from build123d import *

# Parameters (mm, degrees)
SKETCH1_R           = 6
BOSS_EXTRUDE1_DEPTH = 5
SKETCH2_R           = 4
BOSS_EXTRUDE2_DEPTH = 1
SKETCH3_R           = 3
CUT_EXTRUDE1_DEPTH  = 11.392304845
CHAMFER1_SIZE       = 0.2


with BuildPart() as part:
    # Sketch1 → Boss-Extrude1 (new body)
    with BuildSketch(Plane.XY):
        Circle(SKETCH1_R)
    extrude(amount=BOSS_EXTRUDE1_DEPTH)

    # Sketch2 → Boss-Extrude2 (add)
    with BuildSketch(Plane.XY.offset(5)):
        Circle(SKETCH2_R)
    extrude(amount=BOSS_EXTRUDE2_DEPTH)

    # Sketch3 → Cut-Extrude1 (cut, through all)
    with BuildSketch(Plane.XY.offset(6)):
        Circle(SKETCH3_R)
    extrude(amount=-CUT_EXTRUDE1_DEPTH, mode=Mode.SUBTRACT)

    # Chamfer1
    chamfer1_edges = [part.edges().sort_by_distance(p)[0] for p in [
        (-6, 0, 0),
        (-6, 0, 5),
    ]]
    chamfer(chamfer1_edges, length=CHAMFER1_SIZE)

    # Sketch4 → M3 Tapped Hole1 (revolve, cut)
    with BuildSketch(Plane(origin=(0, 0, 2.5), x_dir=(0, 0, -1), z_dir=(1, 0, 0))):
        Polygon((0, 0), (0, 8.251075774), (1.25, 7.5), (1.25, 0), align=None)
    revolve(axis=Axis((0, -6.35, 2.5), (0, 1, 0)), mode=Mode.SUBTRACT)


solid = part.part
Source: CAD feature listing. Evaluate the final solid. Frame: model axes, mm. A direction names the side the tool comes from. Give positions to 0.01 mm unless a question says otherwise; leave off trailing zeros. Loops run counter-clockwise (first coordinate to the right, second up) from the corner with the lowest first, then second, coordinate; pieces in that order, holes last. Notation, with made-up numbers: (36, 64) -> (87, 64) arc R10 ccw to (87, 72) -> close; hole circle Ø4 at (2.25, 86.25). An arc over 180 degrees is marked (long way). Use a Markdown table: item, result. Add a question column.
1) Reachability of faces 4 (the face through (-1.24, 4.34, 2.66)), 5 (the face through (-0.867, -3.905, 5.493)), 6 (the face through (1, 3, 6)) from +Z, -Z, +X, -X, +Y, -Y: full face, straight path, thin tool, end or side. Return the list, or none.
2) First-contact query: pin 1 (1 mm diameter, centred on x = -2.5, z = 1.5, fed in from +Y). Flat tip, straight axial feed; report the tip coordinate or a pass-through.
3) Line query: line 1 along Y through (x, z) = (0, 4.25); line 2 along Z through (x, y) = (0, 3.45); line 3 along Z through (x, y) = (3.5, -2). Output: solid intervals per line, ascending. Write a range as [from, to].
4) Pull-direction query (X, two-part tool) for faces 1 (the face through (-0.65, -2.93, 3.04)), 2 (the face through (-1.301, -5.857, 2.468)), 3 (the face through (2.5, -2.5, 0)); classes: +X half, -X half, draft (parallel to the pull), parting line (faces both ways), or undercut.
5) Section query B-B, the plane y = 0. Return the cut outline in (x, z).
6) Section query C-C, the plane z = 5.5. Return the cut outline in (x, y), then the cut area to 3 significant figures.
7) Section query D-D, the plane z = 2.75. Return the cut outline in (x, y).
8) Section query A-A, the plane x = 0. Return the cut outline in (y, z), then the cut area to 3 significant figures.
Numbers:
| question | item | result |
|---|---|---|
| 1 | face 4 | +Y |
| 1 | face 5 | +Z |
| 1 | face 6 | +Z, +X, -X, +Y, -Y |
| 2 | pin 1 | stops at y = 5.66 |
| 3 | line 1 | y = [-6, -3], [3, 6] |
| 3 | line 2 | z = [0, 1.25], [3.75, 6] |
| 3 | line 3 | z = [0, 5] |
| 4 | face 1 | undercut |
| 4 | face 2 | parting line |
| 4 | face 3 | draft |
| 5 | outline | (-6, 0.2) -> (-5.8, 0) -> (-3, 0) -> (-3, 6) -> (-4, 6) -> (-4, 5) -> (-5.8, 5) -> (-6, 4.8) -> close; (3, 0) -> (5.8, 0) -> (6, 0.2) -> (6, 4.8) -> (5.8, 5) -> (4, 5) -> (4, 6) -> (3, 6) -> close |
| 6 | outline | circle Ø8 at (0, 0); hole circle Ø6 at (0, 0) |
| 6 | area | 22.0 mm2 |
| 7 | outline | (-1.22, 2.74) -> (-1.22, 5.87) arc R6 ccw (long way) to (1.22, 5.87) -> (1.22, 2.74) arc R3 cw (long way) to start |
| 8 | outline | (-6, 0.2) -> (-5.8, 0) -> (-3, 0) -> (-3, 6) -> (-4, 6) -> (-4, 5) -> (-5.8, 5) -> (-6, 4.8) -> close; (3, 0) -> (5.8, 0) -> (6, 0.2) -> (6, 1.25) -> (3, 1.25) -> close; (3, 3.75) -> (6, 3.75) -> (6, 4.8) -> (5.8, 5) -> (4, 5) -> (4, 6) -> (3, 6) -> close |
| 8 | area | 24.4 mm2 |
